Input: part model. Units: mm. Frame: model coordinates. A direction names the side the tool comes from. Give positions to 0.01 mm unless a question says otherwise; leave off trailing zeros. Loops run counter-clockwise (first coordinate to the right, second up) from the corner with the lowest first, then second, coordinate; pieces in that order, holes last. Notation, with made-up numbers: M 32.5,21 L 62.5,21 A21 ccw 62.5,57 Z; hole C 70,57 d6. An arc over 180 degrees is marked long. Use CSV: the item, a comma, the result in double quotes. Start each with the question number.
from build123d import *

# Parameters (mm, degrees)
EXTRUDE_714_DEPTH      = 8
SKETCH_2_2_R           = 23.58
SKETCH_2_2_R_2         = 18
CUT_EXTRUDE_1047_DEPTH = 8
CUT_EXTRUDE_1047_DRAFT = -55
SKETCH_5_R             = 23.569219382
SKETCH_5_R_2           = 18
CUT_EXTRUDE_2_DEPTH    = 6.0502
CUT_EXTRUDE_2_DRAFT    = -55


with BuildPart() as part:
    # Sketch 2 → 旋转1 (revolve)
    with BuildSketch(Plane.XY, mode=Mode.PRIVATE) as revolve_1_sk:
        Polygon((0, 0), (120, 0), (120, 14.5), (119.5, 15), (12.5, 15), (12, 14.5), (0, 14.5), align=None)
    revolve(revolve_1_sk.sketch.rotate(Axis((0, 0, 0), (1, 0, 0)), 90), axis=Axis((0, 0, 0), (1, 0, 0)))

    # Sketch 1 → Extrude 714 (add)
    with BuildSketch(Plane(origin=(0, -0.910076524, 0.397317176), x_dir=(0, 0, 1), z_dir=(-1, 0, 0))):
        Polygon((-21.181926867, 0.910076524), (-10.789622021, -17.089923476), (9.99498767, -17.089923476), (20.387292515, 0.910076524), (9.99498767, 18.910076524), (-10.789622021, 18.910076524), align=None)
    extrude(amount=EXTRUDE_714_DEPTH)


with BuildPart() as cut_extrude_1047_tool:
    # Sketch 2 2 → Cut-Extrude 1047 (with draft: the straight prism first)
    with BuildSketch(Plane.ZY.offset(8)):
        Circle(SKETCH_2_2_R)
        Circle(SKETCH_2_2_R_2, mode=Mode.SUBTRACT)
    extrude(amount=-CUT_EXTRUDE_1047_DEPTH)
    # Cut-Extrude 1047: the draft: its side faces are tilted about the plane it starts from
    cut_extrude_1047_sides = [cut_extrude_1047_tool.faces().sort_by_distance(p)[0] for p in [
        (-4, 0, -23.58),
        (-4, 0, -18),
    ]]
    draft(cut_extrude_1047_sides, Plane.ZY.offset(8), CUT_EXTRUDE_1047_DRAFT)


with BuildPart() as part_1:
    add(part.part)

    # Cut-Extrude 1047: cut by cut_extrude_1047_tool
    add(cut_extrude_1047_tool.part, mode=Mode.SUBTRACT)


with BuildPart() as cut_extrude_2_tool:
    # 草图5 → 切除-拉伸2 (with draft: the straight prism first)
    with BuildSketch(Plane(origin=(0, 0, 0), x_dir=(0, 0, -1), z_dir=(1, 0, 0))):
        Circle(SKETCH_5_R)
        Circle(SKETCH_5_R_2, mode=Mode.SUBTRACT)
    extrude(amount=-CUT_EXTRUDE_2_DEPTH)
    # 切除-拉伸2: the draft: its side faces are tilted about the plane it starts from
    cut_extrude_2_sides = [cut_extrude_2_tool.faces().sort_by_distance(p)[0] for p in [
        (-3.0251, 0, 23.569219382),
        (-3.0251, 0, 18),
    ]]
    draft(cut_extrude_2_sides, Plane(origin=(0, 0, 0), x_dir=(0, 0, -1), z_dir=(1, 0, 0)), CUT_EXTRUDE_2_DRAFT)


with BuildPart() as part_2:
    add(part_1.part)

    # 切除-拉伸2: cut by cut_extrude_2_tool
    add(cut_extrude_2_tool.part, mode=Mode.SUBTRACT)

    # 草图6 → 切除-旋转1 (revolve, cut)
    with BuildSketch(Plane.XY, mode=Mode.PRIVATE) as cut_revolve_1_sk:
        Polygon((0, 0), (120, 0), (120, 8), (-8, 8), (-8, 0), align=None)
    revolve(cut_revolve_1_sk.sketch.rotate(Axis((0, 0, 0), (1, 0, 0)), 90), axis=Axis((0, 0, 0), (1, 0, 0)), mode=Mode.SUBTRACT)


solid = part_2.part
Item 1: Section B-B (x = 41.5). Output: boundary loops of the cut face in (y, z), then the cut area to 3 significant figures.
Item 2: Material intervals for line 1 (Y direction, x = 72.5, z = 0); line 2 (X direction, y = 6, z = -17); line 3 (Y direction, x = 36.5, z = -12), sorted ascending.
Item 3: First-contact query: pin 1 Ø1 at (x, y) = (82.5, -1) entering from +Z; pin 2 Ø8 at (y, z) = (7, -16) entering from +X; pin 3 Ø8 at (x, z) = (101, -7) entering from -Y; pin 4 Ø1.5 at (x, z) = (28, 6.5) entering from -Y. Flat tips, straight axial feed; report the tip coordinate or a pass-through.
Item 4: Mould query, pull axis X, two halves, no side actions, for faces 1 (the conical face through (-7.535, 16.141, 9.371)), 2 (the conical face through (-0.465, 16.141, -9.371)), 3 (the cylindrical face through (5.916, 12.864, 6.691)). Classes: +X half, -X half, draft (parallel to the pull), parting line (faces both ways), or undercut.
Item 5: Set-up query: faces 4 (the cylindrical face through (65.25, -12.65, 8.06)), 5 (the flat face through (0, 15, 1)), 6 (the conical face through (-0.465, -16.186, -9.292)). Return all of +Z, -Z, +X, -X, +Y, -Y with unobstructed straight access to the full face (end or side cutting, diameter ignored); none if empty.
Item 6: Section A-A (x = 4.5). Output: boundary loops of the cut face in (y, z).
Recorded:
1,outline,"C 0,0 d30; hole C 0,0 d16"
1,area,"506 mm²"
2,line 1,"-15 to -8, 8 to 15"
2,line 2,"-7.98 to -0.02"
2,line 3,"-9 to 9"
3,pin 1,"z = 14.99"
3,pin 2,"x = 120"
3,pin 3,"y = -14.7"
3,pin 4,"y = -13.85"
4,face 1,"-X half"
4,face 2,"+X half"
4,face 3,"undercut"
5,face 4,"+X"
5,face 5,"none"
5,face 6,"-Z, +X, -Y"
6,outline,"C 0,0 d29; hole C 0,0 d16"
